Print and shaded views of the part. All mm, measured from the part's lowest x, y and z. A direction names the side the tool comes from. Coordinates: 2 decimals unless noted, no trailing zeros. Order: outer loops, then holes, each group sorted by start corner. A loop starts at its lowest first (then second) coordinate and runs counter-clockwise, first axis right, second up.
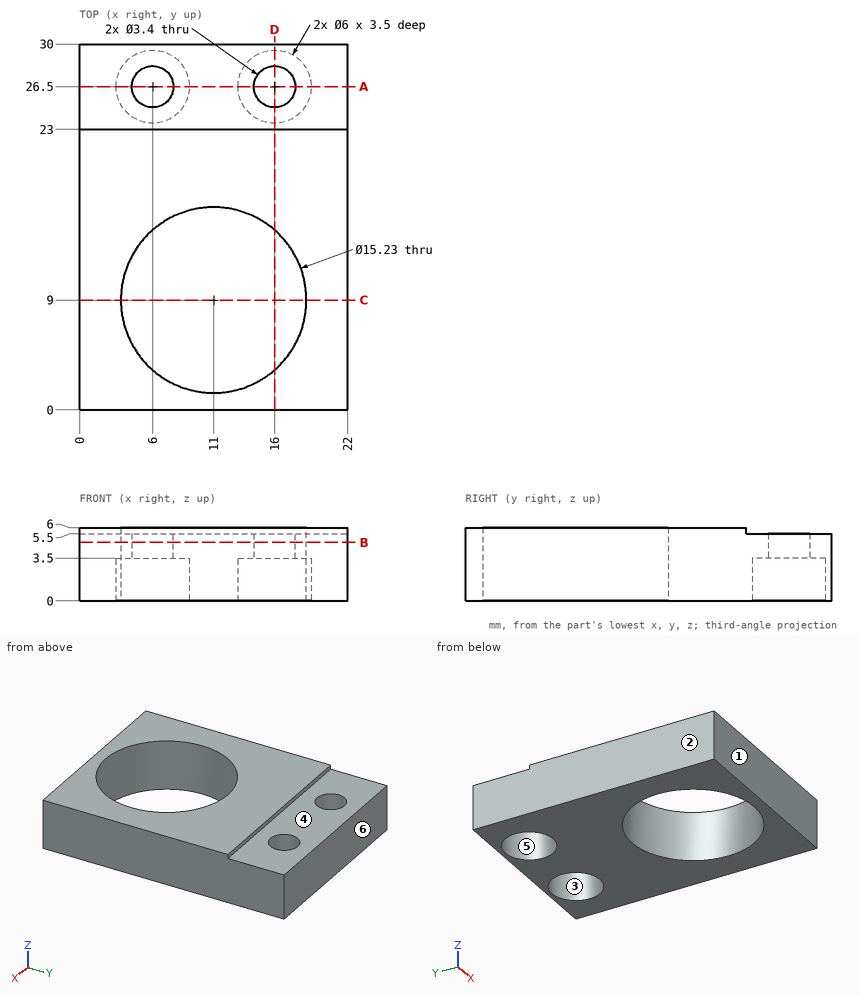
Q1. Mould opens along X. For the marked faces 1, 2 and 3 say: pulls with the +X half, pulls with the -X half, needs draft (parallel to the pull), parting line crosses it, or undercut.
Established:
face 1: needs draft
face 2: pulls with the -X half
face 3: undercut
Q2. Cut at C-C, the plane y = 9. List the corners of the cut face in (x, z) (3 decimals).
Established:
outline: (0, 0) - (3.385, 0) - (3.385, 6) - (0, 6) - close; (18.615, 0) - (22, 0) - (22, 6) - (18.615, 6) - close
Q3. Cut at D-D, the plane x = 16. List the corners of the cut face in (y, z).
Established:
outline: (0, 0) - (3.26, 0) - (3.26, 6) - (0, 6) - close; (14.74, 0) - (23.5, 0) - (23.5, 3.5) - (24.8, 3.5) - (24.8, 5.5) - (23, 5.5) - (23, 6) - (14.74, 6) - close; (28.2, 3.5) - (29.5, 3.5) - (29.5, 0) - (30, 0) - (30, 5.5) - (28.2, 5.5) - close
Q4. Drop flat-ended pins along their axis: P1, Ø1, axis at x = 17.5, y = 18, coming from the -Z side; P2, Ø0.6, axis at x = 14.5, z = 6, coming from the +Y side; P3, Ø3, axis at x = 6, y = 26.5, coming from the +Z side; P4, Ø2, axis at x = 9, y = 25, coming from the +Z side. Give the stop position or say it passes through.
Established:
P1: stops at z = 0
P2: stops at y = 23
P3: passes through
P4: stops at z = 5.5
Q5. Probe line 1 (X direction, y = 26.5, z = 4.15); line 2 (Y direction, x = 11, z = 3.75) (3 decimals); line 3 (Y direction, x = 15.5, z = 5.05). List the from-to ranges inside material, lowest first.
Established:
line 1: x = 0 to 4.3, 7.7 to 14.3, 17.7 to 22
line 2: y = 0 to 1.385, 16.615 to 30
line 3: y = 0 to 2.86, 15.14 to 24.88, 28.12 to 30
Q6. Which spindle directions (+Z, -Z, +X, -X, +Y, -Y) get a long thin tool onto all of the face, cutting with end or side? Do the marked faces 4, 5 and 6. Say none if no direction does.
Established:
face 4: +Z, +X, -X, +Y
face 5: -Z
face 6: +Z, -Z, +X, -X, +Y
Q7. Cut at A-A, the plane y = 26.5. List the corners of the cut face in (x, z), plus the area to 3 significant figures.
Established:
outline: (0, 0) - (3, 0) - (3, 3.5) - (4.3, 3.5) - (4.3, 5.5) - (0, 5.5) - close; (7.7, 3.5) - (9, 3.5) - (9, 0) - (13, 0) - (13, 3.5) - (14.3, 3.5) - (14.3, 5.5) - (7.7, 5.5) - close; (17.7, 3.5) - (19, 3.5) - (19, 0) - (22, 0) - (22, 5.5) - (17.7, 5.5) - close
area: 65.4 mm2
Q8. Cut at B-B, the plane z = 4.8. List the corners of the cut face in (x, y) (3 decimals).
Established:
outline: (0, 0) - (22, 0) - (22, 30) - (0, 30) - close; hole circle Ø15.23 at (11, 9); hole circle Ø3.4 at (6, 26.5); hole circle Ø3.4 at (16, 26.5)
